Can you work these out from the drawing? Everything is in mm from the part's minimum corner. Round coordinates to 2 decimals unless told otherwise and drop trailing zeros. Order: outer loops, then holes, each group sorted by start corner. A loop starts at its lowest first (then second) coordinate and runs counter-clockwise, first axis right, second up. Notation, with made-up numbers: M 48,44 L 96,44 A33 cw 96,72 Z; hole C 87.5,-12 d11. An arc over 180 degrees is marked long. Write each question's results on one line, items separated by ' | '. Start each with the question number.
1. Suppose I cut it at A-A on y = 1.45. Write out the boundary of the cut face in (x, z).
2. We'd pull the mould along Y, two halves only. Please class the marked faces 1 and 2: released by +Y, released by -Y, zero draft, split by the parting line, or undercut.
3. Please list where these lines run through material, in increasing order: L1, parallel to X at y = 1.7, z = 13.5; L2, parallel to X at y = 1.45, z = 16.
4. I'm going to push a flat-ended pin straight in: pin 1 (5 mm diameter, centred on x = 3, z = 17, fed in from -Y). Where does the tip first touch, or does it pass through?
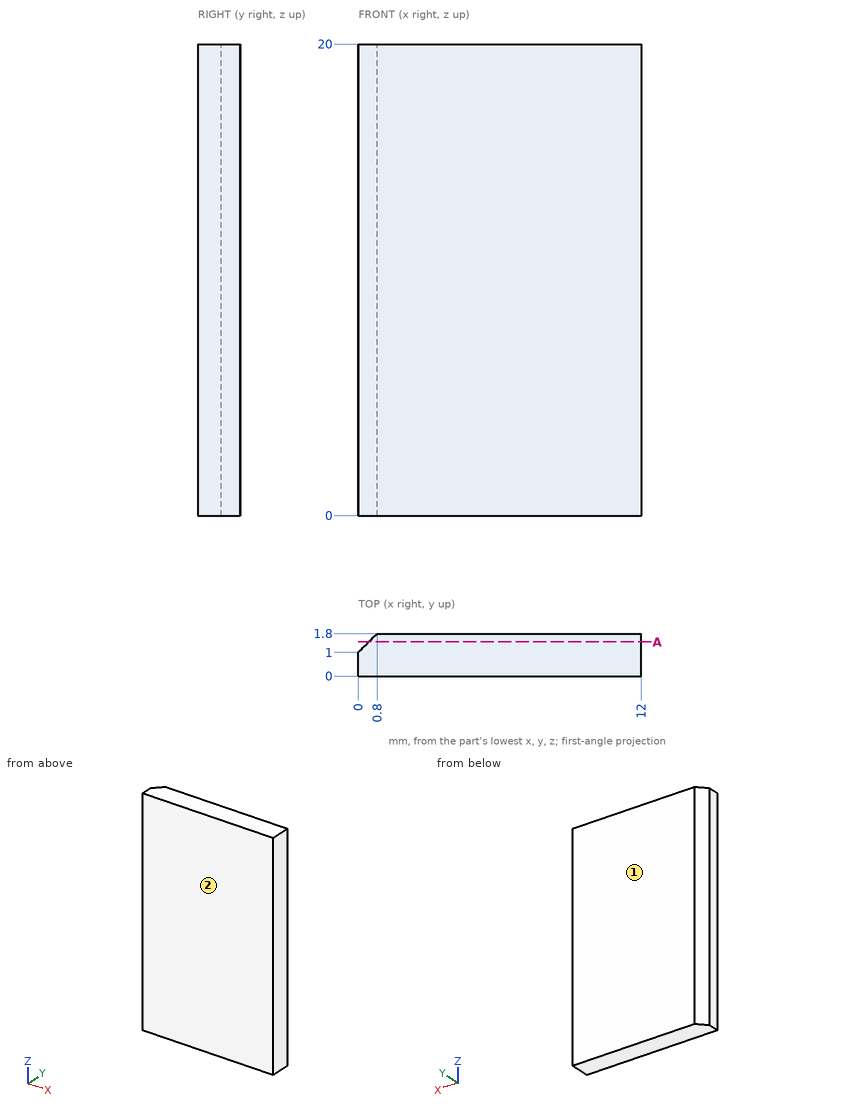
Filled sheet:
1) outline: M 0.45,0 L 12,0 L 12,20 L 0.45,20 Z
2) face 1: released by +Y | face 2: released by -Y
3) L1: x = 0.7 to 12 | L2: x = 0.45 to 12
4) pin 1: stops at y = 0
